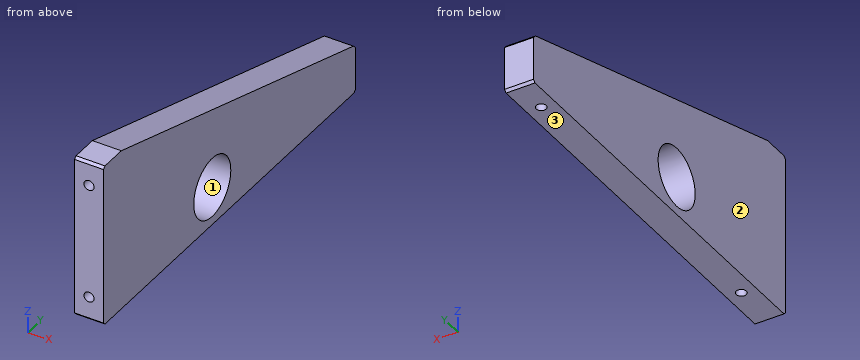
```python
from build123d import *
from OCP.BRepFilletAPI import BRepFilletAPI_MakeChamfer

# Parameters (mm, degrees)
BOSS_EXTRUDE1_DEPTH   = 6
M5_TAPPED_HOLE1_D     = 4.2
M5_TAPPED_HOLE1_DEPTH = 12.4
M5_TAPPED_HOLE1_TIP   = 1.2618073
M5_TAPPED_HOLE2_D     = 4.2
M5_TAPPED_HOLE2_DEPTH = 12.4
M5_TAPPED_HOLE2_TIP   = 1.2618073
CHAMFER1_SIZE         = 1
CHAMFER1_SIZE2        = 1.501184106
SKETCH6_R             = 12.5
CUT_EXTRUDE1_DEPTH    = 184.488419253


with BuildPart() as part:
    # Sketch1 → Boss-Extrude1 (new, symmetric)
    with BuildSketch(Plane(origin=(0, 0, 0), x_dir=(0, 0, -1), z_dir=(1, 0, 0))):
        Polygon((0, 0), (-68, 0), (-68, 12), (-20, 170), (0, 170), align=None)
    extrude(amount=BOSS_EXTRUDE1_DEPTH, both=True)

    # M5 Tapped Hole1
    with Locations(Plane(origin=(0, 0, 0), x_dir=(-1, 0, 0), z_dir=(0, 0, -1))):
        with Locations((0, 20), (0, 155)):
            Hole(M5_TAPPED_HOLE1_D / 2, depth=M5_TAPPED_HOLE1_DEPTH)
            with Locations((0, 0, -(M5_TAPPED_HOLE1_DEPTH + M5_TAPPED_HOLE1_TIP / 2))):  # 118° drill point
                Cone(0, M5_TAPPED_HOLE1_D / 2, M5_TAPPED_HOLE1_TIP, mode=Mode.SUBTRACT)

    # M5 Tapped Hole2
    with Locations(Plane(origin=(0, 0, 0), x_dir=(-1, 0, 0), z_dir=(0, -1, 0))):
        with Locations((0, -58), (0, -10)):
            Hole(M5_TAPPED_HOLE2_D / 2, depth=M5_TAPPED_HOLE2_DEPTH)
            with Locations((0, 0, -(M5_TAPPED_HOLE2_DEPTH + M5_TAPPED_HOLE2_TIP / 2))):  # 118° drill point
                Cone(0, M5_TAPPED_HOLE2_D / 2, M5_TAPPED_HOLE2_TIP, mode=Mode.SUBTRACT)

    # Chamfer1: one chamfer whose edges measure the first distance from different faces: ONE call of the kernel's chamfer builder (chamfer() names one face for all edges)
    chamfer1_edges_1 = [part.edges().sort_by_distance(p)[0] for p in [
        (0, 0, 0),
        (0, 0, 68),
        (0, 170, 0),
    ]]
    chamfer1_edges_2 = [part.edges().sort_by_distance(p)[0] for p in [
        (0, 170, 20),
    ]]
    chamfer1_side_2 = [part.faces().sort_by_distance(p)[0] for p in [
        (0, 170, 10),
    ]]
    chamfer1 = BRepFilletAPI_MakeChamfer(part.part.solid().wrapped)
    for e in chamfer1_edges_1:
        chamfer1.Add(CHAMFER1_SIZE, e.wrapped)
    for e in chamfer1_edges_2:
        chamfer1.Add(CHAMFER1_SIZE, CHAMFER1_SIZE2, e.wrapped, chamfer1_side_2[0].wrapped)  # the first distance lies on this face
    add(Compound.cast(chamfer1.Shape()), mode=Mode.REPLACE)

    # Sketch6 → Cut-Extrude1 (cut, through all)
    with BuildSketch(Plane(origin=(6, 0, 0), x_dir=(0, 0, -1), z_dir=(1, 0, 0))):
        with Locations((-16, 73.4)):
            Circle(SKETCH6_R)
    extrude(amount=-CUT_EXTRUDE1_DEPTH, mode=Mode.SUBTRACT)


solid = part.part
```
Here's how the part is built. I have some questions about the finished solid (model axes, mm). Face numbers are marked on the shaded views. Give positions to 0.01 mm unless a question says otherwise; leave off trailing zeros. Write each loop counter-clockwise with the first axis right and the second up, starting at its lowest first coordinate (ties: lowest second). Pieces come first, ordered by that corner, then holes.
(1) Thinking about a two-plate mould opening in Z: for the marked faces 1, 2 and 3, which applies, pulls with the +Z half, pulls with the -Z half, needs draft (parallel to the pull), parting line crosses it, or undercut?
Output values:
face 1: undercut
face 2: needs draft
face 3: pulls with the -Z half
(2) Imagine slicing it at B-B, the plane y = 73.4. Write out the boundary of the cut face in (x, z).
Output values:
outline: (-6, 0) - (6, 0) - (6, 3.5) - (-6, 3.5) - close; (-6, 28.5) - (6, 28.5) - (6, 49.35) - (-6, 49.35) - close
(3) Will these pins go through, and if not, where does the flat tip stop? pin 1 (2.5 mm diameter, centred on x = 0, y = 155, fed in from +Z); pin 2 (3.5 mm diameter, centred on x = 0, z = 58, fed in from -Y); pin 3 (3 mm diameter, centred on x = -2.5, y = 48, fed in from +Z).
Output values:
pin 1: stops at z = 24.94
pin 2: stops at y = 12.61
pin 3: stops at z = 57.52
(4) If I drill on L1, parallel to Y at x = 0.75, z = 16; L2, parallel to X at y = 9.5, z = 10; L3, parallel to Y at x = -0.5, z = 10, over which ranges is the centre line in solid material (lowest first)?
Output values:
L1: y = 0 to 60.9, 85.9 to 170
L2: x = -6 to -2.1, 2.1 to 6
L3: y = 13.36 to 17.96, 22.04 to 62.43, 84.37 to 152.96, 157.04 to 170
(5) Imagine slicing it at A-A, the plane z = 16. Write out the boundary of the cut face in (x, y).
Output values:
outline: (-6, 0) - (6, 0) - (6, 60.9) - (-6, 60.9) - close; (-6, 85.9) - (6, 85.9) - (6, 170) - (-6, 170) - close
(6) Imagine slicing it at D-D, the plane z = 40.5. Write out the boundary of the cut face in (x, y), and give its area (3 significant figures).
Output values:
outline: (-6, 0) - (6, 0) - (6, 102.52) - (-6, 102.52) - close
area: 1,230 mm2
(7) Imagine slicing it at C-C, the plane y = 91. Write out the boundary of the cut face in (x, z), and give its area (3 significant figures).
Output values:
outline: (-6, 0) - (6, 0) - (6, 44) - (-6, 44) - close
area: 528 mm2
